Verification items for this drawing (mm, ordinates from the low corner). A direction names the side the tool comes from. Give positions to 0.01 mm unless a question says otherwise; leave off trailing zeros. Loops run counter-clockwise (first coordinate to the right, second up) from the corner with the lowest first, then second, coordinate; pieces in that order, holes last. Notation, with made-up numbers: M 50.25,81.25 L 83.25,81.25 A30 ccw 83.25,108.25 Z; hole C -40,-25.75 d8. An arc over 180 degrees is marked long. Use one line per item in the form item = value.
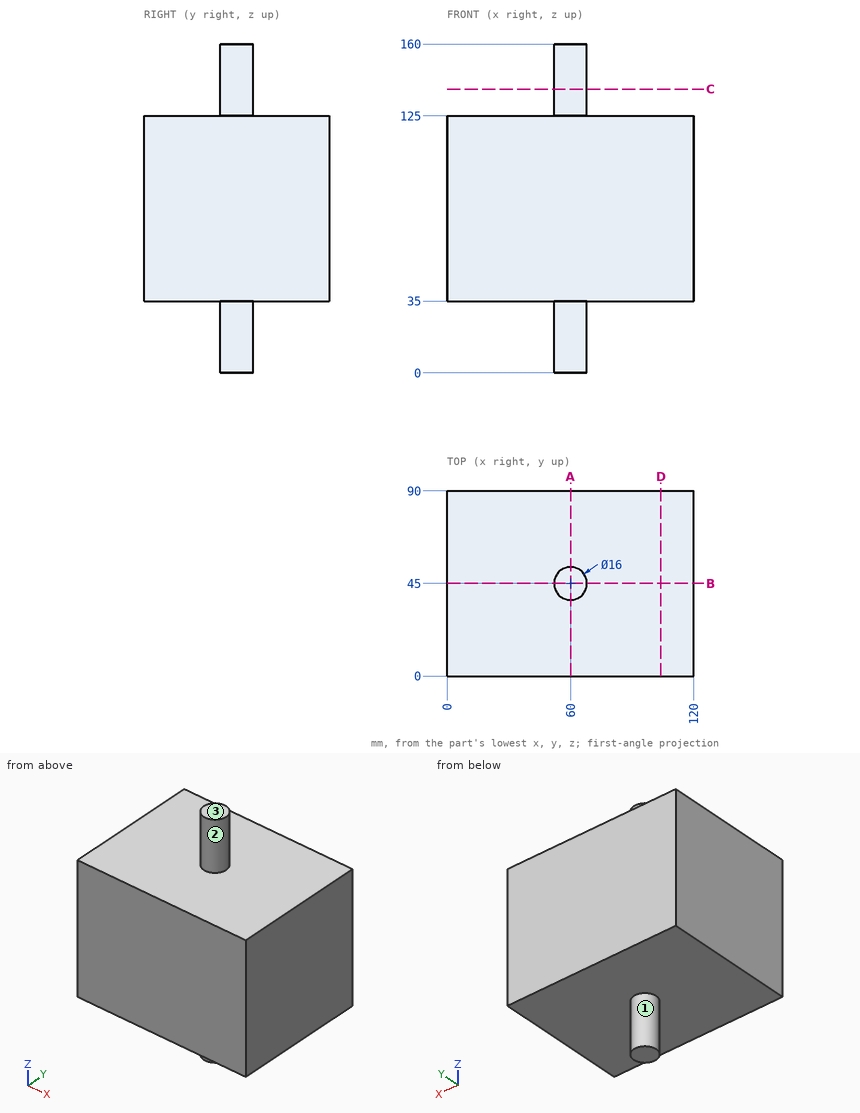
1) Section check C-C (z = 138). Record the cut outline in (x, y), then the cut area to 3 significant figures.
Evaluation:
outline = C 60,45 d16
area = 201 mm^2
2) Set-up check for the marked faces 1, 2 and 3: record each of +Z, -Z, +X, -X, +Y, -Y from which the full face is reachable in a straight line by a thin tool's end or side.
Evaluation:
face_1 = -Z
face_2 = +Z
face_3 = +Z, +X, -X, +Y, -Y
3) Section check D-D (x = 104). Record the cut outline in (y, z).
Evaluation:
outline = M 0,35 L 90,35 L 90,125 L 0,125 Z
4) Depth check by flat-ended pin: pin 1 Ø10 at (y, z) = (36.5, 143) entering from +X; pin 2 Ø10 at (x, y) = (18, 49.5) entering from -Z. Enter the tip coordinate at first touch or a pass-through.
Evaluation:
pin_1 = 67.19
pin_2 = 35
5) Section check A-A (x = 60). Record the cut outline in (y, z), then the cut area to 3 significant figures.
Evaluation:
outline = M 0,35 L 37,35 L 37,0 L 53,0 L 53,35 L 90,35 L 90,125 L 53,125 L 53,160 L 37,160 L 37,125 L 0,125 Z
area = 9,220 mm^2
6) Section check B-B (y = 45). Record the cut outline in (x, z), then the cut area to 3 significant figures.
Evaluation:
outline = M 0,35 L 52,35 L 52,0 L 68,0 L 68,35 L 120,35 L 120,125 L 68,125 L 68,160 L 52,160 L 52,125 L 0,125 Z
area = 11,900 mm^2
7) Scan lines: line 1 (Z direction, x = 91, y = 6); line 2 (Y direction, x = 57, z = 126). Record each from-to range of solid material in increasing order.
Evaluation:
line_1 = 35 to 125
line_2 = 37.58 to 52.42
